Input: part model. Units: mm. Frame: model coordinates. Give positions to 0.01 mm unless a question says otherwise; leave off trailing zeros. Loops run counter-clockwise (first coordinate to the right, second up) from the corner with the lowest first, then second, coordinate; pieces in that order, holes last. Notation, with made-up numbers: M -26,3 L 9,3 A22 ccw 9,26 Z; hole C 36.25,1.5 d3. An arc over 180 degrees is marked long. Answer as a JSON object with one key per item and string values. Group by question number.
```python
from build123d import *

# Parameters (mm, degrees)
SKETCH_1_R      = 8.5
EXTRUDE_1_DEPTH = 70
SKETCH_2_R      = 12.5
EXTRUDE_2_DEPTH = 670
SKETCH_3_R      = 10
EXTRUDE_3_DEPTH = 34
SKETCH_4_R      = 8.5
EXTRUDE_4_DEPTH = 40
CHAMFER_1_SIZE  = 0.5
FILLET_1_R      = 0.3
FILLET_2_R      = 0.3
SKETCH_5_R      = 3
EXTRUDE_5_DEPTH = 20


with BuildPart() as part:
    # 草图1 → 拉伸1 (new body)
    with BuildSketch(Plane(origin=(0, 0, 0), x_dir=(1, 0, 0), z_dir=(0, 1, 0))):
        with Locations(Location((0, 0, 0), (0, 0, 270))):
            Circle(SKETCH_1_R)
    extrude(amount=EXTRUDE_1_DEPTH)

    # 草图2 → 拉伸2 (add)
    with BuildSketch(Plane(origin=(0, 70, 0), x_dir=(-1, 0, 0), z_dir=(0, 1, 0))):
        with Locations(Location((0, 0, 0), (0, 0, 90))):
            Circle(SKETCH_2_R)
    extrude(amount=EXTRUDE_2_DEPTH)

    # 草图3 → 拉伸3 (add)
    with BuildSketch(Plane(origin=(0, 740, 0), x_dir=(-1, 0, 0), z_dir=(0, 1, 0))):
        with Locations(Location((0, 0, 0), (0, 0, 90))):
            Circle(SKETCH_3_R)
    extrude(amount=EXTRUDE_3_DEPTH)

    # 草图4 → 拉伸4 (add)
    with BuildSketch(Plane(origin=(0, 774, 0), x_dir=(-1, 0, 0), z_dir=(0, 1, 0))):
        with Locations(Location((0, 0, 0), (0, 0, 90))):
            Circle(SKETCH_4_R)
    extrude(amount=EXTRUDE_4_DEPTH)

    # 倒角1
    chamfer_1_edges = [part.edges().sort_by_distance(p)[0] for p in [
        (0, 814, -8.5),
        (0, 0, -8.5),
        (0, 70, -12.5),
        (0, 740, -12.5),
    ]]
    chamfer(chamfer_1_edges, length=CHAMFER_1_SIZE)

    # 圆角1
    fillet_1_edges = [part.edges().sort_by_distance(p)[0] for p in [
        (0, 70, -8.5),
    ]]
    fillet(fillet_1_edges, radius=FILLET_1_R)

    # 圆角2
    fillet_2_edges = [part.edges().sort_by_distance(p)[0] for p in [
        (0, 740, -10),
    ]]
    fillet(fillet_2_edges, radius=FILLET_2_R)

    # 草图5 → 拉伸5 (add)
    with BuildSketch(Plane.XZ):
        with Locations(Location((0, 0, 0), (0, 0, 90))):
            Circle(SKETCH_5_R)
    extrude(amount=EXTRUDE_5_DEPTH)


solid = part.part
```
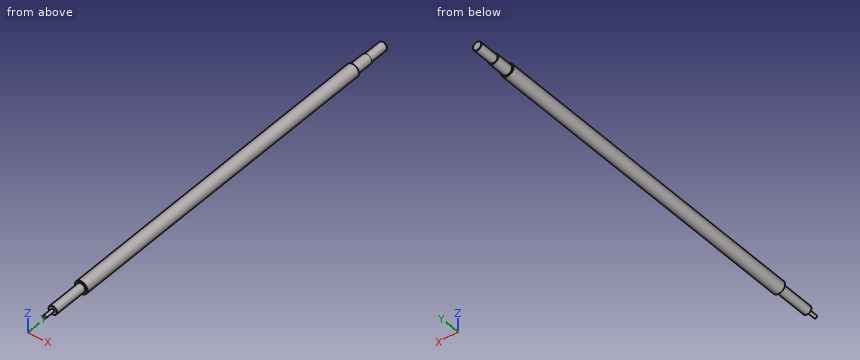
1. First-contact query: P1, Ø6, axis at x = 0.5, y = 230.5, coming from the +Z side; P2, Ø4, axis at y = 630.5, z = 6, coming from the +X side; P3, Ø8, axis at x = 9.5, z = 5, coming from the -Y side; P4, Ø4, axis at y = 362.5, z = 4.5, coming from the -X side. Flat tips, straight axial feed; report the tip coordinate or a pass-through.
2. Section A-A (y = 730). Output: boundary loops of the cut face in (x, z), then the cut area to 3 significant figures.
3. Material intervals for L1, parallel to Z at x = -3.75, y = 466; L2, parallel to Y at x = 5, z = 1.5; L3, parallel to X at y = 390, z = 7, sorted ascending.
Geometry results:
{
 "1": {"P1": "z = 12.5", "P2": "x = 11.84", "P3": "y = 0", "P4": "x = -12.25"},
 "2": {"outline": "C 0,0 d25", "area": "491 mm2"},
 "3": {"L1": "-11.92 to 11.92", "L2": "0 to 814", "L3": "-10.36 to 10.36"}
}
